Could you check a few things on this model? Use its own coordinates, in mm. A direction names the side the tool comes from. Give positions to 0.01 mm unless a question says otherwise; leave off trailing zeros. Write each loop counter-clockwise with the first axis right and the second up, starting at its lowest first coordinate (ties: lowest second). Pieces come first, ordered by that corner, then holes. Notation, with made-up numbers: (23, 34) - (71, 34) arc R28 ccw to (71, 58) - close; hole circle Ø1 at (74, 31.25). An arc over 180 degrees is marked (long way). Answer as CSV lines item,"result". Start each with the question number.
Q1. Imagine slicing it at A-A on z = 0. List the corners of the cut face in (x, y) for me, and give its area (3 significant figures).
Q2. Imagine slicing it at B-B on x = 32. List the corners of the cut face in (y, z) for me.
Q3. Imagine slicing it at D-D on z = 5. List the corners of the cut face in (x, y) for me.
Q4. On a 3-axis mill with a long thin cutter (end or side, diameter ignored), from which of +Z, -Z, +X, -X, +Y, -Y can I reach the whole of each face in a straight line? I mean faces 1 (the face through (4.08, -4, 0)), 2 (the face through (44.08, 0, 0)), 3 (the face through (8.08, -2, 2)), 4 (the face through (5, 4, -1.35)). Say none if no direction works.
Q5. Imagine slicing it at C-C on x = 9.5. List the corners of the cut face in (y, z) for me.
Q6. Will these pins go through, and if not, where does the flat tip stop? pin 1 Ø6 at (x, z) = (8.5, -4) entering from -Y; pin 2 Ø0.7 at (x, y) = (6.5, 3.5) entering from -Z; pin 3 Ø1.1 at (x, y) = (5.5, 4) entering from +Z.
Q7. If I drill on line 1 along X through (y, z) = (-1, -0.5); line 2 along Y through (x, z) = (8, -2.5); line 3 along X through (y, z) = (-0.5, -2.25), over which ranges is the centre line in solid material (lowest first)?
Q8. We'd pull the mould along X, two halves only. Please class faces 5 (the face through (24.257, 1.585, -2.067)), 6 (the face through (5.656, 4.049, -0.019)), 7 (the face through (5, 4, 1.35)): pulls with the +X half, pulls with the -X half, needs draft (parallel to the pull), parting line crosses it, or undercut.
```python
from build123d import *

# Parameters (mm, degrees)
NIB_REACH      = 46.807
SKETCH2_WALL_W = 94.941468098
SKETCH2_WALL_H = 2.7


with BuildPart() as part:
    # Sketch1 → Base (revolve)
    with BuildSketch(Plane.XY, mode=Mode.PRIVATE) as base_sk:
        with BuildLine():
            Line((44.08, 0), (44.08, 3))
            Line((44.08, 3), (8.08, 3))
            Line((8.08, 3), (8.08, 3.24))
            Line((8.08, 3.24), (4.58, 3.24))
            ThreePointArc((4.58, 3.24), (4.226446609, 3.386446609), (4.08, 3.74))
            Line((4.08, 3.74), (4.08, 5.684505256))
            ThreePointArc((4.08, 5.684505256), (1.125576957, 3.498571137), (0, 0))
            Line((0, 0), (44.08, 0))
        make_face()
    revolve(base_sk.sketch.rotate(Axis((-31.484345479, 0, 0), (1, 0, 0)), 90), axis=Axis((-31.484345479, 0, 0), (1, 0, 0)))

    # Sketch2 wall → Nib (add, up to next)
    with BuildSketch(Plane(origin=(5.43, 4.212252628, 0), x_dir=(-0.811462330335, 0.58440472829, 0), z_dir=(-0.58440472829, -0.811462330335, 0)), mode=Mode.PRIVATE) as nib_sk1:
        Rectangle(SKETCH2_WALL_W, SKETCH2_WALL_H)
    nib_tool1 = extrude(nib_sk1.sketch, amount=NIB_REACH, mode=Mode.PRIVATE) - part.part
    add(nib_tool1.solids().sort_by_distance((5.43, 4.212252628, 0))[0])

    # Sketch3 → Cut-Revolve1 (revolve, cut)
    with BuildSketch(Plane.XY, mode=Mode.PRIVATE) as cut_revolve1_sk:
        Polygon((26.08, 3), (23.58, 2.4585), (8.08, 2.4585), (8.08, 3), align=None)
    revolve(cut_revolve1_sk.sketch.rotate(Axis((-29.816341648, 0, 0), (1, 0, 0)), 90), axis=Axis((-29.816341648, 0, 0), (1, 0, 0)), mode=Mode.SUBTRACT)


solid = part.part
```
Conclusion:
1,outline,"(4.08, -5.68) - (4.08, -3.74) arc R0.5 cw to (4.58, -3.24) - (8.08, -3.24) - (8.08, -2.46) - (23.58, -2.46) - (26.08, -3) - (44.08, -3) - (44.08, 3) - (26.08, 3) - (23.58, 2.46) - (8.08, 2.46) - (8.08, 3.24) - (6.78, 3.24) - (4.08, 5.18) - (4.08, 5.68) arc R6 ccw to start"
1,area,"260 mm^2"
2,outline,"circle Ø6 at (0, 0)"
3,outline,"(4.08, -2.7) - (4.08, 2.7) arc R3.32 ccw to start"
4,face 1,"+X"
4,face 2,"+Z, -Z, +X, +Y, -Y"
4,face 3,"none"
4,face 4,"-Z, +X, +Y"
5,outline,"circle Ø4.92 at (0, 0)"
6,pin 1,"y = -3.07"
6,pin 2,"z = -1.35"
6,pin 3,"z = 1.35"
7,line 1,"0.11 to 44.08"
7,line 2,"-2.06 to 2.06"
7,line 3,"0.46 to 44.08"
8,face 5,"undercut"
8,face 6,"pulls with the +X half"
8,face 7,"needs draft"
